CAD build for the part. Positions are in the model's coordinates, mm. A direction names the side the tool comes from. Give positions to 0.01 mm unless a question says otherwise; leave off trailing zeros. Order: outer loops, then holes, each group sorted by start corner. A loop starts at its lowest first (then second) coordinate and runs counter-clockwise, first axis right, second up.
Item 1: Band-saw the part on C-C on z = 2.5. Give the cut face in (x, y), plus the area to 3 significant figures.
Item 2: Two-plate mould, pull along Z, no slides. Class faces 3 (the flat face through (296, 0, 20)), 4 (the flat face through (296, 0, -17)), 5 (the flat face through (296, 37, 0)), 6 (the flat face through (297, -40, 0)): released by +Z, released by -Z, zero draft, split by the parting line, or undercut.
Item 3: Which spindle directions (+Z, -Z, +X, -X, +Y, -Y) get a long thin tool onto all of the face, cutting with end or side? Do faces 1 (the flat face through (296, 40, 0)), 2 (the flat face through (296, 0, 17)). Say none if no direction does.
Item 4: Wall check: L1, parallel to Y at x = 208.5, z = -13.5; L2, parallel to Z at x = 448.5, y = -22; L3, parallel to Y at x = 569, z = -6. Give the ranges that are in metal, low to high.
Item 5: Band-saw the part on A-A on y = 1. Give the cut face in (x, z).
Item 6: Band-saw the part on B-B on x = 164. Give the cut face in (y, z).
```python
from build123d import *

# Parameters (mm, degrees)
COLD_FORMED_RECT_HOLLOW_SECTION_GB_T_672_DEPTH = 600
CUT_EXTRUDE1_DEPTH                             = 603.660766933


with BuildPart() as part:
    # Sketch1 → Cold-Formed Rect Hollow Section GB/T 6728-2002 80 X 40 X 3(1) (new body)
    with BuildSketch(Plane(origin=(0, 0, 0), x_dir=(0, 0, -1), z_dir=(1, 0, 0))):
        with BuildLine():
            Line((-14, -40), (14, -40))
            ThreePointArc((14, -40), (18.242640687, -38.242640687), (20, -34))
            Line((20, -34), (20, 34))
            ThreePointArc((20, 34), (18.242640687, 38.242640687), (14, 40))
            Line((14, 40), (-14, 40))
            ThreePointArc((-14, 40), (-18.242640687, 38.242640687), (-20, 34))
            Line((-20, 34), (-20, -34))
            ThreePointArc((-20, -34), (-18.242640687, -38.242640687), (-14, -40))
        make_face()
        with BuildLine():
            Line((-14, -37), (14, -37))
            ThreePointArc((14, -37), (16.121320344, -36.121320344), (17, -34))
            Line((17, -34), (17, 34))
            ThreePointArc((17, 34), (16.121320344, 36.121320344), (14, 37))
            Line((14, 37), (-14, 37))
            ThreePointArc((-14, 37), (-16.121320344, 36.121320344), (-17, 34))
            Line((-17, 34), (-17, -34))
            ThreePointArc((-17, -34), (-16.121320344, -36.121320344), (-14, -37))
        make_face(mode=Mode.SUBTRACT)
    extrude(amount=COLD_FORMED_RECT_HOLLOW_SECTION_GB_T_672_DEPTH)

    # Sketch2 → Cut-Extrude1 (cut, through all)
    with BuildSketch(Plane.XY.offset(20)):
        Polygon((74, -34), (6, 34), (0, 34), (0, -34), align=None)
        Polygon((600, 34), (594, 34), (526, -34), (600, -34), align=None)
        Polygon((600, -34), (526, -34), (520, -40), (600, -40), align=None)
        Polygon((6, 34), (0, 40), (0, 34), align=None)
        Polygon((600, 40), (594, 34), (600, 34), align=None)
        Polygon((80, -40), (74, -34), (0, -34), (0, -40), align=None)
    extrude(amount=-CUT_EXTRUDE1_DEPTH, mode=Mode.SUBTRACT)


solid = part.part
```
The answers:
1. outline: (0, 40) - (3, 37) - (597, 37) - (600, 40) - close; (77, -37) - (80, -40) - (520, -40) - (523, -37) - close
1. area: 3,120 mm2
2. face 3: released by +Z
2. face 4: undercut
2. face 5: undercut
2. face 6: zero draft
3. face 1: +Z, -Z, +X, -X, +Y
3. face 2: +X, -X
4. L1: y = -40 to -37, 37 to 40
4. L2: z = -20 to -17, 17 to 20
4. L3: y = 37 to 40
5. outline: (39, -20) - (561, -20) - (561, -17) - (39, -17) - close; (39, 17) - (561, 17) - (561, 20) - (39, 20) - close
6. outline: (-40, -14) arc R6 ccw to (-34, -20) - (34, -20) arc R6 ccw to (40, -14) - (40, 14) arc R6 ccw to (34, 20) - (-34, 20) arc R6 ccw to (-40, 14) - close; hole (-37, -14) arc R3 ccw to (-34, -17) - (34, -17) arc R3 ccw to (37, -14) - (37, 14) arc R3 ccw to (34, 17) - (-34, 17) arc R3 ccw to (-37, 14) - close
